Can you work these out from the model? Positions are in its coordinate system, mm. Round coordinates to 2 decimals unless told otherwise and drop trailing zeros. Loops run counter-clockwise (first coordinate to the right, second up) from the corner with the lowest first, then second, coordinate; pieces in that order, holes last. Notation, with made-up numbers: (64, 82) -> (89, 82) arc R14 ccw to (89, 91) -> close; hole circle Ø10 at (6, -16). An arc over 180 degrees is marked (long way). Write item = value, one per line.
from build123d import *

# Parameters (mm, degrees)
SKETCH1_R          = 7
BASE_EXTRUDE_DEPTH = 11
SKETCH2_OUTSIDE_W  = 318.108
SKETCH2_OUTSIDE_H  = 314.706
SKETCH2_OUTSIDE_R  = 10.998522628
CUT_EXTRUDE1_DEPTH = 38
CUT_EXTRUDE1_DRAFT = -75
SKETCH3_OUTSIDE_W  = 318.108
SKETCH3_OUTSIDE_H  = 314.706
SKETCH3_OUTSIDE_R  = 10.998522628
CUT_EXTRUDE2_DEPTH = 38
CUT_EXTRUDE2_DRAFT = -75


with BuildPart() as part:
    # Sketch1 → Base-Extrude (new body)
    with BuildSketch(Plane.XY):
        Polygon((6.35, 10.998522628), (-6.35, 10.998522628), (-12.7, 0), (-6.35, -10.998522628), (6.35, -10.998522628), (12.7, 0), align=None)
        Circle(SKETCH1_R, mode=Mode.SUBTRACT)
    extrude(amount=BASE_EXTRUDE_DEPTH)


with BuildPart() as cut_extrude1_tool:
    # Sketch2 outside → Cut-Extrude1 (with draft: the straight prism first)
    with BuildSketch(Plane(origin=(0, 0, 0), x_dir=(-1, 0, 0), z_dir=(0, 0, -1))):
        Rectangle(SKETCH2_OUTSIDE_W, SKETCH2_OUTSIDE_H)
        Circle(SKETCH2_OUTSIDE_R, mode=Mode.SUBTRACT)
    extrude(amount=-CUT_EXTRUDE1_DEPTH)
    # Cut-Extrude1: the draft: its side faces are tilted about the plane it starts from
    cut_extrude1_sides = [cut_extrude1_tool.faces().sort_by_distance(p)[0] for p in [
        (0, -157.353, 19),
        (-159.054, 0, 19),
        (0, 157.353, 19),
        (159.054, 0, 19),
        (10.998522628, 0, 19),
    ]]
    draft(cut_extrude1_sides, Plane(origin=(0, 0, 0), x_dir=(-1, 0, 0), z_dir=(0, 0, -1)), CUT_EXTRUDE1_DRAFT)


with BuildPart() as part_1:
    add(part.part)

    # Cut-Extrude1: cut by cut_extrude1_tool
    add(cut_extrude1_tool.part, mode=Mode.SUBTRACT)


with BuildPart() as cut_extrude2_tool:
    # Sketch3 outside → Cut-Extrude2 (with draft: the straight prism first)
    with BuildSketch(Plane.XY.offset(11)):
        Rectangle(SKETCH3_OUTSIDE_W, SKETCH3_OUTSIDE_H)
        Circle(SKETCH3_OUTSIDE_R, mode=Mode.SUBTRACT)
    extrude(amount=-CUT_EXTRUDE2_DEPTH)
    # Cut-Extrude2: the draft: its side faces are tilted about the plane it starts from
    cut_extrude2_sides = [cut_extrude2_tool.faces().sort_by_distance(p)[0] for p in [
        (0, -157.353, -8),
        (159.054, 0, -8),
        (0, 157.353, -8),
        (-159.054, 0, -8),
        (-10.998522628, 0, -8),
    ]]
    draft(cut_extrude2_sides, Plane.XY.offset(11), CUT_EXTRUDE2_DRAFT)


with BuildPart() as part_2:
    add(part_1.part)

    # Cut-Extrude2: cut by cut_extrude2_tool
    add(cut_extrude2_tool.part, mode=Mode.SUBTRACT)


solid = part_2.part
1. I'm going to push flat-ended pins straight in: pin 1 (6 mm diameter, centred on y = 5.5, z = 7, fed in from -X); pin 2 (1 mm diameter, centred on x = -5.5, y = -2, fed in from -Z); pin 3 (1 mm diameter, centred on y = -7, z = 9, fed in from +X). Where does each tip first touch, or does it pass through?
Entries:
pin_1 = -11.26
pin_2 = through
pin_3 = 8.95
2. We'd pull the mould along Y, two halves only. Please class faces 1 (the flat face through (-9.48, 5.58, 5.42)), 2 (the conical face through (5.68, -9.89, 10.89)), 3 (the cylindrical face through (6.466, -2.681, 5.423)): released by +Y, released by -Y, zero draft, split by the parting line, or undercut.
Entries:
face_1 = released by +Y
face_2 = released by -Y
face_3 = undercut
3. Suppose I cut it at A-A, the plane z = 9.5. List the corners of the cut face in (x, y) for me, and give its area (3 significant figures).
Entries:
outline = (-12.7, 0) -> (-6.35, -11) -> (6.35, -11) -> (12.7, 0) -> (6.35, 11) -> (-6.35, 11) -> close; hole circle Ø14 at (0, 0)
area = 265 mm²
4. I need wall thicknesses on line 1 (Y direction, x = -0.25, z = 7.25); line 2 (Y direction, x = -5.75, z = 10); line 3 (X direction, y = -3.75, z = 8). Which ranges of each line are inside material? Lowest first, please. Write a range as [from, to].
Entries:
line_1 = [-11, -7], [7, 11]
line_2 = [-11, -3.99], [3.99, 11]
line_3 = [-10.53, -5.91], [5.91, 10.53]
